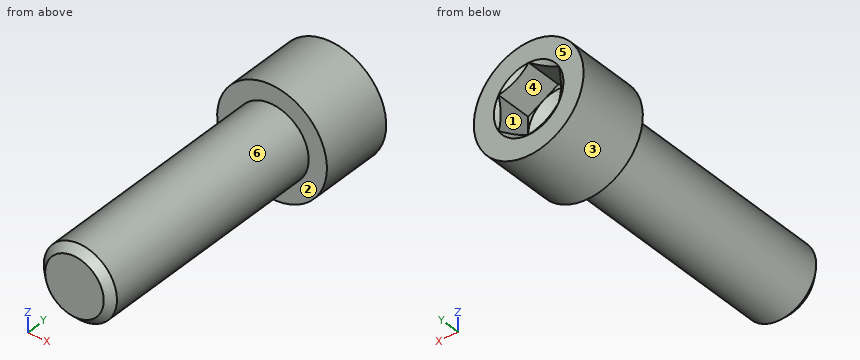
```python
from build123d import *

# Parameters (mm, degrees)
SKETCH1_R           = 9
BOSS_EXTRUDE1_DEPTH = 12
SKETCH2_R           = 6
BOSS_EXTRUDE2_DEPTH = 40
CUT_EXTRUDE1_DEPTH  = 6
CHAMFER1_SIZE       = 1.2


with BuildPart() as part:
    # Sketch1 → Boss-Extrude1 (new body)
    with BuildSketch(Plane(origin=(0, 0, 0), x_dir=(1, 0, 0), z_dir=(0, 1, 0))):
        with Locations(Location((0, 0, 0), (0, 0, 270))):
            Circle(SKETCH1_R)
    extrude(amount=BOSS_EXTRUDE1_DEPTH)

    # Sketch2 → Boss-Extrude2 (add)
    with BuildSketch(Plane.XZ):
        with Locations(Location((0, 0, 0), (0, 0, 90))):
            Circle(SKETCH2_R)
    extrude(amount=BOSS_EXTRUDE2_DEPTH)

    # Sketch3 → Cut-Extrude1 (cut)
    with BuildSketch(Plane(origin=(0, 12, 0), x_dir=(1, 0, 0), z_dir=(0, 1, 0))):
        Polygon((0, 5.7), (-4.936344802, 2.85), (-4.936344802, -2.85), (0, -5.7), (4.936344802, -2.85), (4.936344802, 2.85), align=None)
    extrude(amount=-CUT_EXTRUDE1_DEPTH, mode=Mode.SUBTRACT)

    # Sketch4 → Cut-Revolve1 (revolve, cut)
    with BuildSketch(Plane.XY, mode=Mode.PRIVATE) as cut_revolve1_sk:
        Polygon((0, 6), (4.936344802, 6), (0, 3.15), align=None)
        Polygon((4.936344802, 11.559103466), (4.936344802, 12), (5.7, 12), align=None)
    revolve(cut_revolve1_sk.sketch.rotate(Axis((0, -3.932195077, 0), (0, 1, 0)), 270), axis=Axis((0, -3.932195077, 0), (0, 1, 0)), mode=Mode.SUBTRACT)

    # Chamfer1
    chamfer1_edges = [part.edges().sort_by_distance(p)[0] for p in [
        (0, -40, -6),
    ]]
    chamfer(chamfer1_edges, length=CHAMFER1_SIZE)


solid = part.part
```
Geometry check sheet. Reference: the model listing, model coordinates, mm. Face numbers are marked on the shaded views. A direction names the side the tool comes from. Give positions to 0.01 mm unless a question says otherwise; leave off trailing zeros. Write each loop counter-clockwise with the first axis right and the second up, starting at its lowest first coordinate (ties: lowest second). Pieces come first, ordered by that corner, then holes. Notation, with made-up numbers: (-13.75, 39) - (32.25, 39) arc R23 ccw to (32.25, 54) - close; hole circle Ø1 at (7.25, -33). An arc over 180 degrees is marked (long way). Use a Markdown table: item, result.
Q1. Thickness scan on L1, parallel to Y at x = 4.5, z = 6.25; L2, parallel to X at y = -19, z = 0.25; L3, parallel to Y at x = -3.75, z = 3.5. Record the ranges inside material, lowest first. Write a range as [from, to].
Computed:
| item | result |
|---|---|
| L1 | y = [0, 12] |
| L2 | x = [-5.99, 5.99] |
| L3 | y = [-39.67, 6] |
Q2. Section check B-B, the plane z = -6.5. Enter the section's corners in (x, y).
Computed:
| item | result |
|---|---|
| outline | (-6.22, 0) - (6.22, 0) - (6.22, 12) - (-6.22, 12) - close |
Q3. Go/stop test with flat-tipped pins: P1, Ø5, axis at y = -10.5, z = -0.5, coming from the -X side; P2, Ø2, axis at x = -0.5, y = -11, coming from the +Z side; P3, Ø1.1, axis at x = -1, z = 5, coming from the +Y side. Record where each tip stops, or that it passes through.
Computed:
| item | result |
|---|---|
| P1 | stops at x = -6 |
| P2 | stops at z = 6 |
| P3 | stops at y = 11.97 |
Q4. Draft check along Z on the marked faces 4, 5 and 6. Enter one of: pulls with the +Z half, pulls with the -Z half, needs draft (parallel to the pull), parting line crosses it, or undercut.
Computed:
| item | result |
|---|---|
| face 4 | undercut |
| face 5 | needs draft |
| face 6 | parting line crosses it |
Q5. Section check A-A, the plane y = -25. Enter the section's corners in (x, z), then the cut area to 3 significant figures.
Computed:
| item | result |
|---|---|
| outline | circle Ø12 at (0, 0) |
| area | 113 mm² |
Q6. Section check C-C, the plane x = 7.25. Enter the section's corners in (y, z), then the cut area to 3 significant figures.
Computed:
| item | result |
|---|---|
| outline | (0, -5.33) - (12, -5.33) - (12, 5.33) - (0, 5.33) - close |
| area | 128 mm² |
Q7. Set-up check for the marked faces 1, 2 and 3: record each of +Z, -Z, +X, -X, +Y, -Y from which the full face is reachable in a straight line by a thin tool's end or side.
Computed:
| item | result |
|---|---|
| face 1 | +Y |
| face 2 | -Y |
| face 3 | +Y, -Y |
